Part model, mm, in its own coordinate system. Face numbers are marked on the shaded views. A direction names the side the tool comes from. Give positions to 0.01 mm unless a question says otherwise; leave off trailing zeros. Write each loop counter-clockwise with the first axis right and the second up, starting at its lowest first coordinate (ties: lowest second). Pieces come first, ordered by that corner, then holes. Notation, with made-up numbers: M 88,-31 L 128,-31 A27 ccw 128,-3 Z; hole C 59,81.5 d1. An arc over 180 degrees is marked long. Use CSV: the item, a comma, the result in double quotes. Start each with the question number.
1. Band-saw the part on C-C, the plane z = -31. List the corners of the cut face in (x, y).
2. 3-axis set-ups, long thin cutter, end or side, ignore diameter. For the marked faces 1 and 2: which of +Z, -Z, +X, -X, +Y, -Y reach the whole face in a straight line?
3. Band-saw the part on B-B, the plane x = 11. List the corners of the cut face in (y, z).
4. Drop flat-ended pins along their axis: pin 1 Ø3 at (y, z) = (-8.5, 31) entering from -X; pin 2 Ø1.5 at (x, z) = (-6.5, -4.5) entering from +Y; pin 3 Ø8 at (x, y) = (0, 0) entering from +Z. Give the stop position or say it passes through.
5. Drill centre lines: line 1 along Y through (x, z) = (0, -59); line 2 along Y through (x, z) = (0, -71); line 3 along Z through (x, y) = (15.5, -5.5). Where is each one in solid material? Low to high. Write a range as from..to.
6. Band-saw the part on A-A, the plane z = 66.5. List the corners of the cut face in (x, y), then the cut area to 3 significant figures.
from build123d import *

# Parameters (mm, degrees)
SKETCH1_R              = 15
BOSS_EXTRUDE1_DEPTH    = 68
SKETCH2_R              = 12.5
BOSS_EXTRUDE2_DEPTH    = 15
BOSS_EXTRUDE4_START    = 25
SKETCH4_R              = 17.5
BOSS_EXTRUDE4_DEPTH    = 3
M12_TAPPED_HOLE1_D     = 10.2
M12_TAPPED_HOLE1_DEPTH = 32.75
M12_TAPPED_HOLE1_TIP   = 3.064389157
M12_TAPPED_HOLE2_D     = 10.2
M12_TAPPED_HOLE2_DEPTH = 32.75
M12_TAPPED_HOLE2_TIP   = 3.064389157


with BuildPart() as part:
    # Sketch1 → Boss-Extrude1 (new, symmetric)
    with BuildSketch(Plane.XY):
        Circle(SKETCH1_R)
    extrude(amount=BOSS_EXTRUDE1_DEPTH, both=True)

    # Sketch2 → Boss-Extrude2 (add)
    with BuildSketch(Plane.XY.offset(68)):
        Circle(SKETCH2_R)
    boss_extrude2 = extrude(amount=BOSS_EXTRUDE2_DEPTH)

    # Mirror1: Boss-Extrude2 across plane
    add(boss_extrude2.mirror(Plane.XY))

    # Sketch4 → Boss-Extrude4 (add)
    with BuildSketch(Plane.XY.offset(BOSS_EXTRUDE4_START)):
        Circle(SKETCH4_R)
    extrude(amount=BOSS_EXTRUDE4_DEPTH)

    # M12 Tapped Hole1
    with Locations(Plane(origin=(0, 0, -83), x_dir=(-1, 0, 0), z_dir=(0, 0, -1))):
        with Locations((0, 0)):
            Hole(M12_TAPPED_HOLE1_D / 2, depth=M12_TAPPED_HOLE1_DEPTH)
            with Locations((0, 0, -(M12_TAPPED_HOLE1_DEPTH + M12_TAPPED_HOLE1_TIP / 2))):  # 118° drill point
                Cone(0, M12_TAPPED_HOLE1_D / 2, M12_TAPPED_HOLE1_TIP, mode=Mode.SUBTRACT)

    # M12 Tapped Hole2
    with Locations(Plane.XY.offset(83)):
        with Locations((0, 0)):
            Hole(M12_TAPPED_HOLE2_D / 2, depth=M12_TAPPED_HOLE2_DEPTH)
            with Locations((0, 0, -(M12_TAPPED_HOLE2_DEPTH + M12_TAPPED_HOLE2_TIP / 2))):  # 118° drill point
                Cone(0, M12_TAPPED_HOLE2_D / 2, M12_TAPPED_HOLE2_TIP, mode=Mode.SUBTRACT)


solid = part.part
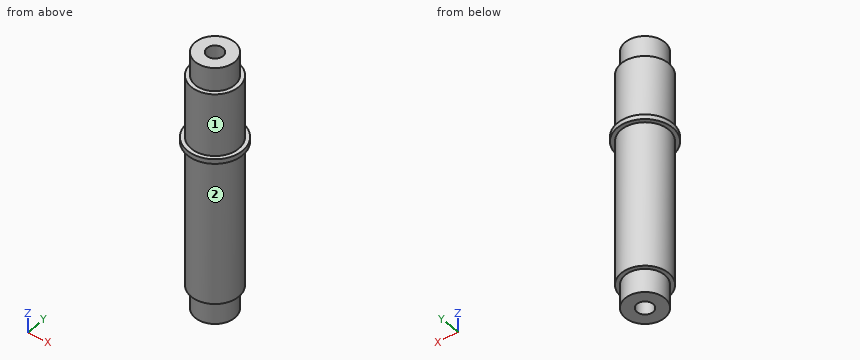
Output:
1,outline,"C 0,0 d30"
2,face 1,"+Z"
2,face 2,"-Z"
3,outline,"M -13.61,25 L -10.2,25 L -10.2,-68 L -5.94,-68 L -5.94,-83 L 5.94,-83 L 5.94,-68 L 10.2,-68 L 10.2,25 L 13.61,25 L 13.61,28 L 10.2,28 L 10.2,68 L 5.94,68 L 5.94,83 L -5.94,83 L -5.94,68 L -10.2,68 L -10.2,28 L -13.61,28 Z"
4,pin 1,"stops at x = -13.27"
4,pin 2,"stops at y = 13.85"
4,pin 3,"stops at z = 49.59"
5,line 1,"y = -15..-5.1, 5.1..15"
5,line 2,"y = -12.5..-5.1, 5.1..12.5"
5,line 3,"z = 25..28"
6,outline,"C 0,0 d30; hole C 0,0 d10.2"
6,area,"625 mm²"
